from build123d import *

# Parameters (mm, degrees)
SKETCH1_W           = 70
SKETCH1_H           = 100
BOSS_EXTRUDE1_DEPTH = 30
SKETCH2_R           = 4
BOSS_EXTRUDE2_DEPTH = 4
SKETCH3_R           = 10
BOSS_EXTRUDE3_DEPTH = 50
SKETCH4_W           = 70
SKETCH4_H           = 100
BOSS_EXTRUDE4_DEPTH = 15
SKETCH5_W           = 134.250739562
SKETCH5_H           = 64.864054132
CUT_EXTRUDE1_DEPTH  = 130
CUT_EXTRUDE2_REACH  = 189.566
SKETCH6_W           = 60
SKETCH6_H           = 6
SKETCH7_W           = 100
SKETCH7_H           = 39
BOSS_EXTRUDE5_DEPTH = 60


with BuildPart() as part:
    # Sketch1 → Boss-Extrude1 (new body)
    with BuildSketch(Plane(origin=(0, 0, 0), x_dir=(1, 0, 0), z_dir=(0, 1, 0))):
        Rectangle(SKETCH1_W, SKETCH1_H)
    extrude(amount=BOSS_EXTRUDE1_DEPTH)

    # Sketch2 → Boss-Extrude2 (add)
    # profile 1 of 3: a face of its own
    with BuildSketch(Plane(origin=(0, 30, 0), x_dir=(1, 0, 0), z_dir=(0, 1, 0))):
        with Locations(Location((20, -35, 0), (0, 0, 270))):
            Circle(SKETCH2_R)
        Polygon((21.913058762, -37.035169602), (22.719037957, -34.360827314), (20.805979195, -32.325657712), (18.086941238, -32.964830398), (17.280962043, -35.639172686), (19.194020805, -37.674342288), align=None, mode=Mode.SUBTRACT)
    # profile 2 of 3: a face of its own
    with BuildSketch(Plane(origin=(0, 30, 0), x_dir=(1, 0, 0), z_dir=(0, 1, 0))):
        with Locations(Location((20, 0, 0), (0, 0, 270))):
            Circle(SKETCH2_R)
        Polygon((21.913058762, -1.47020522), (22.229764451, 0.921654877), (20.316705689, 2.391860097), (18.086941238, 1.47020522), (17.770235549, -0.921654877), (19.683294311, -2.391860097), align=None, mode=Mode.SUBTRACT)
    # profile 3 of 3: a face of its own
    with BuildSketch(Plane(origin=(0, 30, 0), x_dir=(1, 0, 0), z_dir=(0, 1, 0))):
        with Locations(Location((20, 35, 0), (0, 0, 270))):
            Circle(SKETCH2_R)
        Polygon((21.913058762, 33.534680981), (22.225532876, 35.924097978), (20.312474114, 37.389416996), (18.086941238, 36.465319019), (17.774467124, 34.075902022), (19.687525886, 32.610583004), align=None, mode=Mode.SUBTRACT)
    extrude(amount=BOSS_EXTRUDE2_DEPTH)

    # Sketch3 → Boss-Extrude3 (add)
    with BuildSketch(Plane(origin=(35, 0, 0), x_dir=(0, 0, -1), z_dir=(1, 0, 0))):
        Circle(SKETCH3_R)
    extrude(amount=BOSS_EXTRUDE3_DEPTH)

    # Sketch4 → Boss-Extrude4 (add)
    with BuildSketch(Plane.XZ):
        Rectangle(SKETCH4_W, SKETCH4_H)
    extrude(amount=BOSS_EXTRUDE4_DEPTH)

    # Mirror1: part across plane


with BuildPart() as part_1:
    add(part.part)
    add(part.part.mirror(Plane(origin=(-35, 30, -50), x_dir=(0, 0, 1), z_dir=(1, 0, 0))))

    # Sketch5 → Cut-Extrude1 (cut)
    with BuildSketch(Plane.ZY.offset(35)):
        with Locations((0.773607985, 10.636315649)):
            Rectangle(SKETCH5_W, SKETCH5_H)
    extrude(amount=-CUT_EXTRUDE1_DEPTH, mode=Mode.SUBTRACT)

    # Sketch6 → Cut-Extrude2 (cut, up to next)
    with BuildSketch(Plane.XY.offset(50), mode=Mode.PRIVATE) as cut_extrude2_sk1:
        with Locations((-65, -12)):
            Rectangle(SKETCH6_W, SKETCH6_H)
    cut_extrude2_tool1 = extrude(cut_extrude2_sk1.sketch, amount=-CUT_EXTRUDE2_REACH, mode=Mode.PRIVATE) & part_1.part
    add(cut_extrude2_tool1.solids().sort_by_distance((-65, -12, 50))[0], mode=Mode.SUBTRACT)

    # Sketch7 → Boss-Extrude5 (add)
    with BuildSketch(Plane(origin=(-35, 0, 0), x_dir=(0, 0, -1), z_dir=(1, 0, 0))):
        with Locations((0, 10.5)):
            Rectangle(SKETCH7_W, SKETCH7_H)
    extrude(amount=BOSS_EXTRUDE5_DEPTH)


solid = part_1.part
Work out the finished part from the listing and answer in its coordinate system (mm). A direction names the side the tool comes from. Coordinates: 2 decimals unless noted, no trailing zeros. Write each loop counter-clockwise with the first axis right and the second up, starting at its lowest first coordinate (ties: lowest second). Pieces come first, ordered by that corner, then holes. Notation, with made-up numbers: M 83,37.5 L 113,37.5 A14 ccw 113,61.5 Z; hole C 14.5,45.5 d6. An arc over 180 degrees is marked long. Answer as CSV lines item,"result". Start each with the question number.
Item 1: Flat-ended cylindrical pins translate along their axes: P1, Ø1.3, axis at x = -90.5, z = -0.5, coming from the +Y side; P2, Ø1.8, axis at y = -13.5, z = -7, coming from the +X side; P3, Ø4, axis at y = 24, z = -24, coming from the -X side. Find the tip coordinate at first contact, or state that the pin passes through.
Item 2: Consider L1, parallel to Y at x = 7, z = -44; L2, parallel to Y at x = -107, z = 0; L3, parallel to X at y = 19, z = 0. Determine where each line is inside the solid, lowest interval first.
Item 3: A tool of negligible diameter and unlimited length cuts with its end or side. For faces 1 (the face through (-129.65, -9.76, 2.17)), 2 (the face through (-95, -12, 1)), 3 (the face through (-86.095, 31.972, -35.867)), from which of +Z, -Z, +X, -X, +Y, -Y can it reach the whole face along a straight path? Write none if from no direction.
Item 4: Section D-D on z = 6.5 is taken. Write down the section's boundary in (x, y).
Item 5: Section B-B on y = 0 is taken. Write down the section's boundary in (x, z), and give its area (3 significant figures).
Item 6: Section A-A on z = -42 is taken. Write down the section's boundary in (x, y), and give its area (3 significant figures).
Item 7: Section C-C on x = 7 is taken. Write down the section's boundary in (y, z), and give its area (3 significant figures).
Checks:
1,P1,"stops at y = 30"
1,P2,"stops at x = -95"
1,P3,"stops at x = -105"
2,L1,"y = -9 to 30"
2,L2,"y = -10 to 10"
2,L3,"x = -105 to 25"
3,face 1,"-X"
3,face 2,"+Z, -Z, +X, -Y"
3,face 3,"+Y"
4,outline,"M -155,-7.6 L -105,-7.6 L -105,-15 L -95,-15 L -95,-9 L 25,-9 L 25,30 L -105,30 L -105,7.6 L -155,7.6 Z"
5,outline,"M -155,-10 L -105,-10 L -105,-50 L 25,-50 L 25,50 L -105,50 L -105,10 L -155,10 Z"
5,area,"14,000 mm²"
6,outline,"M -105,-15 L -95,-15 L -95,-9 L 25,-9 L 25,30 L -105,30 Z"
6,area,"5,130 mm²"
7,outline,"M -9,-50 L 30,-50 L 30,50 L -9,50 Z"
7,area,"3,900 mm²"
